Check sheet for the drawn part. Datum: minimum x, y, z corner. Units: mm. A direction names the side the tool comes from. Round coordinates to 2 decimals unless told otherwise and drop trailing zeros. Write each loop counter-clockwise with the first axis right and the second up, starting at its lowest first coordinate (ties: lowest second). Pieces come first, ordered by that corner, then holes. Notation, with made-up numbers: M 39.25,-39.5 L 79.25,-39.5 A26 cw 79.25,-7.5 Z; hole C 14,84 d10. An arc over 180 degrees is marked long. One line per item, written item: value. Start each with the question number.
1. Section check C-C (z = 5). Record the boundary of the cut face in (x, y).
2. Scan lines: probe 1 along Y at (x, z) = (5, 4.55); probe 2 along Y at (x, z) = (3.75, 7.5); probe 3 along X at (y, z) = (104, 5.35). Record each from-to range of solid material in increasing order. Write a range as [from, to].
3. Depth check by flat-ended pin: P1, Ø2.5, axis at x = 4, z = 1, coming from the +Y side; P2, Ø4.5, axis at x = 4, y = 3, coming from the -Z side; P3, Ø1.5, axis at x = 4, z = 2, coming from the -Y side. Enter the tip coordinate at first touch or a pass-through.
4. Section check A-A (x = 5). Record the boundary of the cut face in (y, z), and give its area (3 significant figures).
5. Access from +Z, -Z, +X, -X, +Y, -Y to the whole of each face (thin tool, end or side, straight path). Record for the marked faces 4 and 5.
6. Section check D-D (y = 20). Record the boundary of the cut face in (x, z).
7. Section check B-B (y = 6). Record the boundary of the cut face in (x, z), and give its area (3 significant figures).
8. Release check for a two-part mould opening along Z. For the marked faces 1, 2 and 3 record: pulls with the +Z half, pulls with the -Z half, needs draft (parallel to the pull), parting line crosses it, or undercut.
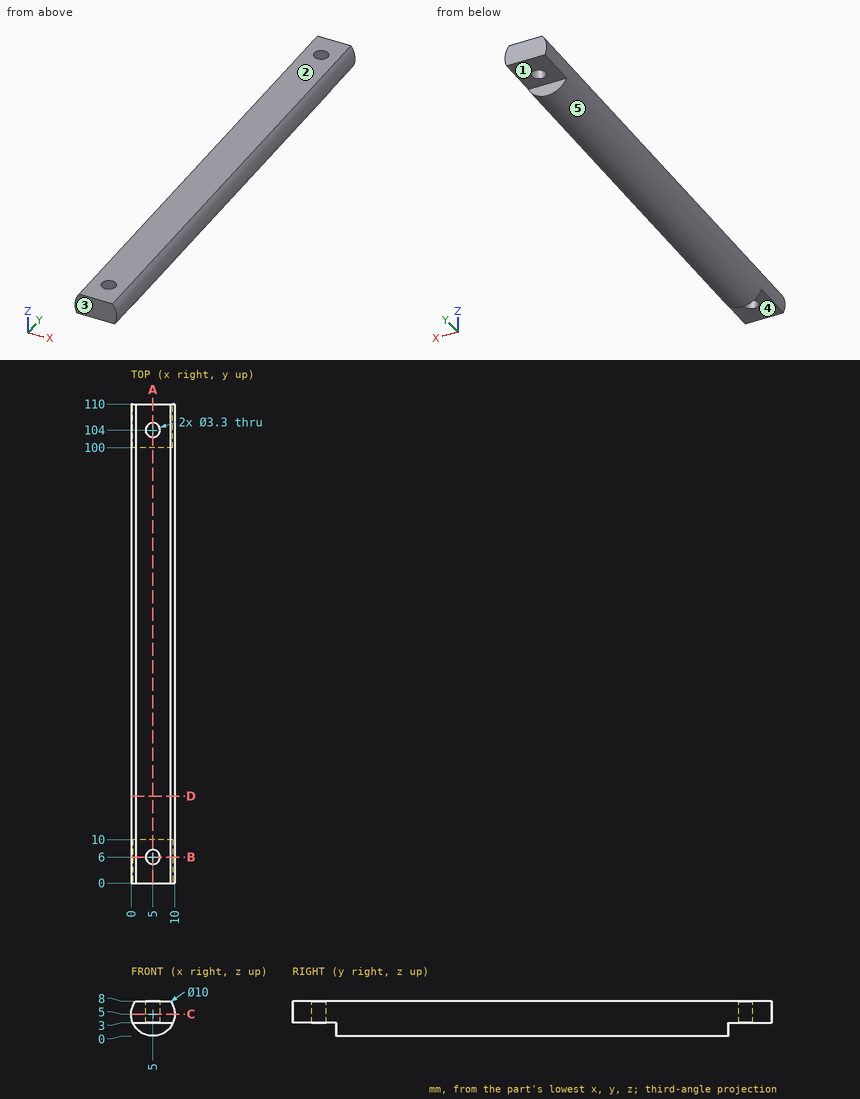
Result sheet:
1. outline: M 0,0 L 10,0 L 10,110 L 0,110 Z; hole C 5,6 d3.3; hole C 5,104 d3.3
2. probe 1: y = [0, 4.35], [7.65, 102.35], [105.65, 110]
2. probe 2: y = [0, 4.92], [7.08, 102.92], [105.08, 110]
2. probe 3: x = [0.01, 3.35], [6.65, 9.99]
3. P1: stops at y = 100
3. P2: stops at z = 3
3. P3: stops at y = 10
4. outline: M 0,3 L 4.35,3 L 4.35,8 L 0,8 Z; M 7.65,3 L 10,3 L 10,0 L 100,0 L 100,3 L 102.35,3 L 102.35,8 L 7.65,8 Z; M 105.65,3 L 110,3 L 110,8 L 105.65,8 Z
4. area: 787 mm2
5. face 4: -Z, +X, -X, -Y
5. face 5: +Y, -Y
6. outline: M 1,8 A5 ccw long 9,8 Z
7. outline: M 0.42,3 L 3.35,3 L 3.35,8 L 1,8 A5 ccw Z; M 6.65,3 L 9.58,3 A5 ccw 9,8 L 6.65,8 Z
7. area: 31.0 mm2
8. face 1: pulls with the -Z half
8. face 2: pulls with the +Z half
8. face 3: needs draft
